Source: CAD feature listing. Evaluate the final solid. Frame: model axes, mm. A direction names the side the tool comes from. Round coordinates to 2 decimals unless told otherwise and drop trailing zeros. Loops run counter-clockwise (first coordinate to the right, second up) from the corner with the lowest first, then second, coordinate; pieces in that order, holes last.
Item 1: Pull-direction query (X, two-part tool) for faces 4 (the flat face through (0, 10, 22.5)), 5 (the cylindrical face through (-8.785, 9.079, -29.636)), 6 (the flat face through (-12.5, -3, 0)); classes: released by +X, released by -X, zero draft, split by the parting line, or undercut.
Item 2: First-contact query: P1, Ø7.5, axis at x = -2.5, z = 7, coming from the +Y side; P2, Ø5, axis at x = 0.5, z = -28, coming from the +Y side; P3, Ø1.8, axis at x = -0.5, z = 16.5, coming from the -Y side. Flat tips, straight axial feed; report the tip coordinate or a pass-through.
Item 3: Section query B-B on y = 6. Return loops of the section in (x, z), then the cut area to 3 significant figures.
Item 4: Ray query, L1, parallel to Z at x = 0, y = -11.75; L2, parallel to Z at x = 0, y = 7; L3, parallel to X at y = 9, z = -28. Return the intervals inside material, ascending.
Item 5: Section query A-A on y = -0.7. Return loops of the section in (x, z), then the cut area to 3 significant figures.
Item 6: Access query for faces 1 (the cylindrical face through (9.215, 9.079, -29.636)), 2 (the flat face through (0, -7.2, 15)), 3 (the flat face through (0, 0, -34)). Directions: +Z, -Z, +X, -X, +Y, -Y. A direction counts if a zero-diameter tool reaches every point of the face in a straight line with its end or side. Return the directions, or none.
Item 7: Section query C-C on z = 15. Return loops of the section in (x, y), then the cut area to 3 significant figures.
Item 8: Section query D-D on x = 5.75. Return loops of the section in (y, z), then the cut area to 3 significant figures.
```python
from build123d import *

# Parameters (mm, degrees)
SKETCH_1_W                   = 25
SKETCH_1_H                   = 68
EXTRUDE_1_DEPTH              = 14.2
CUT_EXTRUDE_1_DEPTH          = 47.030533345
CUT_EXTRUDE_1_DEPTH_BACK     = 10
SKETCH_2_W                   = 25
SKETCH_2_H                   = 45
F_6_0MM_1_D                  = 6
F_6_0MM_1_DEPTH              = 7
HOLE_WIZARD_M5_1_D           = 5.5
HOLE_WIZARD_M5_1_CBORE_D     = 10
HOLE_WIZARD_M5_1_CBORE_DEPTH = 20
HOLE_WIZARD_M4_1_D           = 3.3
HOLE_WIZARD_M4_1_DEPTH       = 10.1
HOLE_WIZARD_M4_1_TIP         = 0.991420021
CHAMFER_1_SIZE               = 1
SKETCH_9_R                   = 4
CUT_EXTRUDE_2_DEPTH          = 45.526845835
SKETCH_10_R                  = 1
CUT_EXTRUDE_3_DEPTH          = 45.526845835


with BuildPart() as part:
    # 草图1 → 凸台-拉伸1 (new, symmetric)
    with BuildSketch(Plane(origin=(0, 0, 0), x_dir=(1, 0, 0), z_dir=(0, 1, 0))):
        Rectangle(SKETCH_1_W, SKETCH_1_H)
    extrude(amount=EXTRUDE_1_DEPTH, both=True)

    # 草图2 → 切除-拉伸1 (cut, two sides: drawn at the far end of the back side and taken through both)
    with BuildSketch(Plane(origin=(0, 14.2, 0), x_dir=(1, 0, 0), z_dir=(0, 1, 0)).offset(-CUT_EXTRUDE_1_DEPTH_BACK)):
        Rectangle(SKETCH_2_W, SKETCH_2_H)
    extrude(amount=CUT_EXTRUDE_1_DEPTH + CUT_EXTRUDE_1_DEPTH_BACK, mode=Mode.SUBTRACT)

    # Ø6.0mm 暗销孔1
    with Locations(Plane(origin=(0, -14.2, 0), x_dir=(-1, 0, 0), z_dir=(0, -1, 0))):
        with Locations((0, 15), (0, -15)):
            Hole(F_6_0MM_1_D / 2, depth=F_6_0MM_1_DEPTH)

    # M5 六角凹头螺钉的柱形沉头孔1 (through all)
    with Locations(Plane(origin=(0, 14.2, 0), x_dir=(1, 0, 0), z_dir=(0, 1, 0))):
        with Locations((0, 28), (0, -28)):
            CounterBoreHole(HOLE_WIZARD_M5_1_D / 2, HOLE_WIZARD_M5_1_CBORE_D / 2, HOLE_WIZARD_M5_1_CBORE_DEPTH)

    # M4 螺纹孔1
    with Locations(Plane(origin=(0, 14.2, 0), x_dir=(1, 0, 0), z_dir=(0, 1, 0))):
        with Locations((-9, -28), (9, -28), (9, 28), (-9, 28)):
            Hole(HOLE_WIZARD_M4_1_D / 2, depth=HOLE_WIZARD_M4_1_DEPTH)
            with Locations((0, 0, -(HOLE_WIZARD_M4_1_DEPTH + HOLE_WIZARD_M4_1_TIP / 2))):  # 118° drill point
                Cone(0, HOLE_WIZARD_M4_1_D / 2, HOLE_WIZARD_M4_1_TIP, mode=Mode.SUBTRACT)

    # 倒角1
    chamfer_1_edges = [part.edges().sort_by_distance(p)[0] for p in [
        (12.5, 0, 34),
        (-12.5, 0, 34),
        (-12.5, 0, -34),
        (12.5, 0, -34),
    ]]
    chamfer(chamfer_1_edges, length=CHAMFER_1_SIZE)

    # 草图9 → 切除-拉伸2 (cut, through all)
    with BuildSketch(Plane.ZY.offset(12.5)):
        with Locations((-12, -0.7)):
            Circle(SKETCH_9_R)
    extrude(amount=-CUT_EXTRUDE_2_DEPTH, mode=Mode.SUBTRACT)

    # 草图10 → 切除-拉伸3 (cut, through all)
    with BuildSketch(Plane(origin=(12.5, 0, 0), x_dir=(0, 0, -1), z_dir=(1, 0, 0))):
        with Locations((-22.5, 4.2)):
            Circle(SKETCH_10_R)
        with Locations((22.5, 4.2)):
            Circle(SKETCH_10_R)
    extrude(amount=-CUT_EXTRUDE_3_DEPTH, mode=Mode.SUBTRACT)


solid = part.part
```
Data:
1. face 4: zero draft
1. face 5: undercut
1. face 6: released by -X
2. P1: stops at y = 4.2
2. P2: stops at y = -5.8
2. P3: stops at y = -7.2
3. outline: (-12.5, -33) - (-11.5, -34) - (11.5, -34) - (12.5, -33) - (12.5, -22.5) - (-12.5, -22.5) - close; (-12.5, 22.5) - (12.5, 22.5) - (12.5, 33) - (11.5, 34) - (-11.5, 34) - (-12.5, 33) - close; hole circle Ø3.3 at (-9, -28); hole circle Ø3.3 at (-9, 28); hole circle Ø10 at (0, -28); hole circle Ø10 at (0, 28); hole circle Ø3.3 at (9, -28); hole circle Ø3.3 at (9, 28)
3. area: 382 mm2
4. L1: z = -34 to -30.75, -25.25 to -18, -12 to 12, 18 to 25.25, 30.75 to 34
4. L2: z = -34 to -33, -23 to -22.5, 22.5 to 23, 33 to 34
4. L3: x = -12.5 to -10.65, -7.35 to -5, 5 to 7.35, 10.65 to 12.5
5. outline: (-12.5, -33) - (-11.5, -34) - (11.5, -34) - (12.5, -33) - (12.5, -16) - (-12.5, -16) - close; (-12.5, -8) - (12.5, -8) - (12.5, 33) - (11.5, 34) - (-11.5, 34) - (-12.5, 33) - close; hole circle Ø10 at (0, -28); hole circle Ø10 at (0, 28)
5. area: 1,340 mm2
6. face 1: +Y
6. face 2: -Y
6. face 3: -Z, +X, -X, +Y, -Y
7. outline: (-12.5, -14.2) - (-3, -14.2) - (-3, -7.2) - (3, -7.2) - (3, -14.2) - (12.5, -14.2) - (12.5, 4.2) - (-12.5, 4.2) - close
7. area: 418 mm2
8. outline: (-14.2, -34) - (14.2, -34) - (14.2, -22.5) - (5.2, -22.5) arc R1 cw (long way) to (4.2, -21.5) - (4.2, 21.5) arc R1 cw (long way) to (5.2, 22.5) - (14.2, 22.5) - (14.2, 34) - (-14.2, 34) - close; hole circle Ø8 at (-0.7, -12)
8. area: 1,430 mm2
